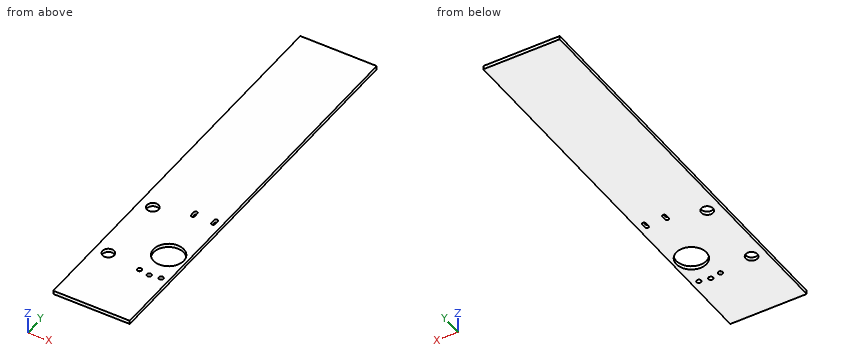
from build123d import *

# Parameters (mm, degrees)
SKETCH_1_W      = 85
SKETCH_1_H      = 445
SKETCH_1_R      = 6.5
SKETCH_1_R_2    = 2.5
SKETCH_1_R_3    = 16.75
EXTRUDE_2_DEPTH = 4


with BuildPart() as part:
    # 草图1 → 凸台-拉伸2 (new body)
    with BuildSketch(Plane.XY):
        with Locations((42.5, -222.5)):
            Rectangle(SKETCH_1_W, SKETCH_1_H)
        with Locations((15, -370)):
            Circle(SKETCH_1_R, mode=Mode.SUBTRACT)
        with Locations((76.970705016, -375.389241728)):
            Circle(SKETCH_1_R_2, mode=Mode.SUBTRACT)
        with Locations((65, -377.5)):
            Circle(SKETCH_1_R_2, mode=Mode.SUBTRACT)
        with Locations((15, -290)):
            Circle(SKETCH_1_R, mode=Mode.SUBTRACT)
        with Locations((53.029294983, -375.389241728)):
            Circle(SKETCH_1_R_2, mode=Mode.SUBTRACT)
        with Locations((65, -342.5)):
            Circle(SKETCH_1_R_3, mode=Mode.SUBTRACT)
        with BuildLine():
            Line((78.3, -275.5), (78.3, -280.5))
            ThreePointArc((78.3, -280.5), (76.3, -282.5), (74.3, -280.5))
            Line((74.3, -280.5), (74.3, -275.5))
            ThreePointArc((74.3, -275.5), (76.3, -273.5), (78.3, -275.5))
        make_face(mode=Mode.SUBTRACT)
        with BuildLine():
            Line((55.8, -275.5), (55.8, -280.5))
            ThreePointArc((55.8, -280.5), (53.8, -282.5), (51.8, -280.5))
            Line((51.8, -280.5), (51.8, -275.5))
            ThreePointArc((51.8, -275.5), (53.8, -273.5), (55.8, -275.5))
        make_face(mode=Mode.SUBTRACT)
    extrude(amount=EXTRUDE_2_DEPTH)


solid = part.part
Geometry check sheet. Reference: the model listing, model coordinates, mm. Give positions to 0.01 mm unless a question says otherwise; leave off trailing zeros. Write each loop counter-clockwise with the first axis right and the second up, starting at its lowest first coordinate (ties: lowest second). Pieces come first, ordered by that corner, then holes. Notation, with made-up numbers: M 13.5,-31 L 50.5,-31 A27 ccw 50.5,-9 Z; hole C 62,69 d8. An arc over 180 degrees is marked long. One line per question, with ' | ' between items.
1. Cross-section at B-B (y = -290). Enter the section's corners in (x, z), plus the area to 3 significant figures.
Ans:
outline: M 0,0 L 8.5,0 L 8.5,4 L 0,4 Z; M 21.5,0 L 85,0 L 85,4 L 21.5,4 Z | area: 288 mm2
2. Gauge pin test, flat ends, axial feed: pin 1 (2 mm diameter, centred on y = -277.5, z = 1.5, fed in from -X); pin 2 (4 mm diameter, centred on x = 53.03, y = -375.39, fed in from +Z). Record the tip position at first contact, or that the pin passes through.
Ans:
pin 1: x = 0 | pin 2: through
3. Scan lines: line 1 along Y through (x, z) = (15, 2.05); line 2 along Y through (x, z) = (65, 1.9); line 3 along Y through (x, z) = (76.5, 2.75). Record each from-to range of solid material in increasing order. Write a range as from..to.
Ans:
line 1: -445..-376.5, -363.5..-296.5, -283.5..0 | line 2: -445..-380, -375..-359.25, -325.75..0 | line 3: -445..-377.84, -372.93..-354.68, -330.32..-282.49, -273.51..0
4. Cross-section at D-D (y = -342.5). Enter the section's corners in (x, z), plus the area to 3 significant figures.
Ans:
outline: M 0,0 L 48.25,0 L 48.25,4 L 0,4 Z; M 81.75,0 L 85,0 L 85,4 L 81.75,4 Z | area: 206 mm2
5. Cross-section at A-A (x = 15). Enter the section's corners in (y, z), plus the area to 3 significant figures.
Ans:
outline: M -445,0 L -376.5,0 L -376.5,4 L -445,4 Z; M -363.5,0 L -296.5,0 L -296.5,4 L -363.5,4 Z; M -283.5,0 L 0,0 L 0,4 L -283.5,4 Z | area: 1,680 mm2
6. Cross-section at C-C (z = 2.6). Count the separate pieces of the cut face and the enclosed holes in it, plus the area to 3 significant figures.
Ans:
separate pieces: 1 | enclosed holes: 8 | area: 36,600 mm2
